```python
from build123d import *

# Parameters (mm, degrees)
BOSS_EXTRUDE1_DEPTH = 3
CUT_EXTRUDE1_DEPTH  = 3
CHAMFER1_SIZE       = 1


with BuildPart() as part:
    # Sketch1 → Boss-Extrude1 (new body)
    with BuildSketch(Plane.XY):
        Polygon((0, 0), (45, 0), (45, 20), (37, 20), (37, 8), (0, 8), align=None)
    extrude(amount=BOSS_EXTRUDE1_DEPTH)

    # Sketch2 → Cut-Extrude1 (cut)
    with BuildSketch(Plane(origin=(0, 0, 0), x_dir=(-1, 0, 0), z_dir=(0, 0, -1))):
        with BuildLine():
            Line((-37, 6), (-33, 6))
            ThreePointArc((-33, 6), (-31, 4), (-33, 2))
            Line((-33, 2), (-37, 2))
            ThreePointArc((-37, 2), (-39, 4), (-37, 6))
        make_face()
        with BuildLine():
            Line((-12, 6), (-8, 6))
            ThreePointArc((-8, 6), (-6, 4), (-8, 2))
            Line((-8, 2), (-12, 2))
            ThreePointArc((-12, 2), (-14, 4), (-12, 6))
        make_face()
    extrude(amount=-CUT_EXTRUDE1_DEPTH, mode=Mode.SUBTRACT)

    # Chamfer1
    chamfer1_edges = [part.edges().sort_by_distance(p)[0] for p in [
        (0, 8, 1.5),
        (37, 20, 1.5),
        (45, 20, 1.5),
        (45, 0, 1.5),
        (0, 0, 1.5),
    ]]
    chamfer(chamfer1_edges, length=CHAMFER1_SIZE)


solid = part.part
```
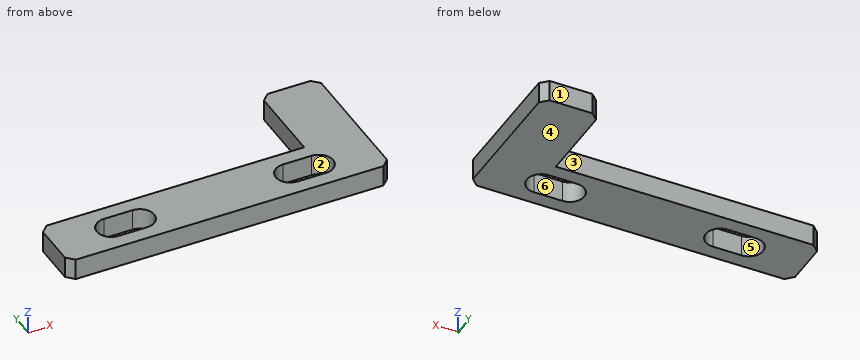
Read the model definition and answer for the solid it produces. Units are mm, in the model's axes. Face numbers are marked on the shaded views. A direction names the side the tool comes from. Coordinates: 2 decimals unless noted, no trailing zeros. Write each loop counter-clockwise with the first axis right and the second up, starting at its lowest first coordinate (ties: lowest second). Pieces come first, ordered by that corner, then holes. Notation, with made-up numbers: (36.25, 17) - (62.25, 17) arc R13 ccw to (62.25, 42) - close; hole circle Ø5 at (-18, 58). An arc over 180 degrees is marked (long way). Answer as a JSON object with one key per item and string values. Group by question number.
1. Consider L1, parallel to X at y = 2.25, z = 1.95; L2, parallel to Y at x = 10.5, z = 2.55; L3, parallel to X at y = 12.25, z = 0.3. Determine where each line is inside the solid, lowest interval first. Write a range as [from, to].
2. A cutting plane is placed at D-D (x = 19). Determine the outline of the cut face in (y, z), plus the area to 3 significant figures.
3. A cutting plane is placed at A-A (y = 4). Determine the outline of the cut face in (x, z).
4. The mould has two halves that part along Y. Classify the marked faces 3, 4, 5 and 6: +Y half, -Y half, draft (parallel to the pull), parting line (faces both ways), or undercut.
5. Which of the six approach directions +Z, -Z, +X, -X, +Y, -Y give full straight-line access (tool end or side, diameter ignored) to the marked faces 1 and 2?
6. A cutting plane is placed at B-B (z = 1.35). Determine the outline of the cut face in (x, y), plus the area to 3 significant figures.
7. A cutting plane is placed at C-C (y = 14.5). Determine the outline of the cut face in (x, z).
8. Each of these flat-tipped pins is pushed along its axis until it touches: P1, Ø1.5, axis at x = 10, z = 1, coming from the +Y side; P2, Ø6, axis at x = 23, y = 11.5, coming from the +Z side. Where does it stop, or does it pass through?
Worked out:
{
 "1": {"L1": "x = [0, 7.03], [12.97, 32.03], [37.97, 45]", "L2": "y = [0, 2], [6, 8]", "L3": "x = [37, 45]"},
 "2": {"outline": "(0, 0) - (8, 0) - (8, 3) - (0, 3) - close", "area": "24.0 mm²"},
 "3": {"outline": "(0, 0) - (6, 0) - (6, 3) - (0, 3) - close; (14, 0) - (31, 0) - (31, 3) - (14, 3) - close; (39, 0) - (45, 0) - (45, 3) - (39, 3) - close"},
 "4": {"face 3": "+Y half", "face 4": "draft", "face 5": "undercut", "face 6": "undercut"},
 "5": {"face 1": "+Z, -Z, +X, -X, +Y", "face 2": "+Z, -Z"},
 "6": {"outline": "(0, 1) - (1, 0) - (44, 0) - (45, 1) - (45, 19) - (44, 20) - (38, 20) - (37, 19) - (37, 8) - (1, 8) - (0, 7) - close; hole (8, 2) - (12, 2) arc R2 ccw to (12, 6) - (8, 6) arc R2 ccw to start; hole (33, 2) - (37, 2) arc R2 ccw to (37, 6) - (33, 6) arc R2 ccw to start", "area": "396 mm²"},
 "7": {"outline": "(37, 0) - (45, 0) - (45, 3) - (37, 3) - close"},
 "8": {"P1": "stops at y = 8", "P2": "passes through"}
}
